Geometry check sheet. Reference: drawing and pictorial views, mm from the part's lowest x, y, z. A direction names the side the tool comes from. Round coordinates to 2 decimals unless told otherwise and drop trailing zeros. Loops run counter-clockwise (first coordinate to the right, second up) from the corner with the lowest first, then second, coordinate; pieces in that order, holes last. Notation, with made-up numbers: (-33.75, 74) -> (-29.75, 74) arc R26 ccw to (-29.75, 103) -> close; hole circle Ø9 at (6.25, 79.5). An arc over 180 degrees is marked (long way). Write item = value, one per line.
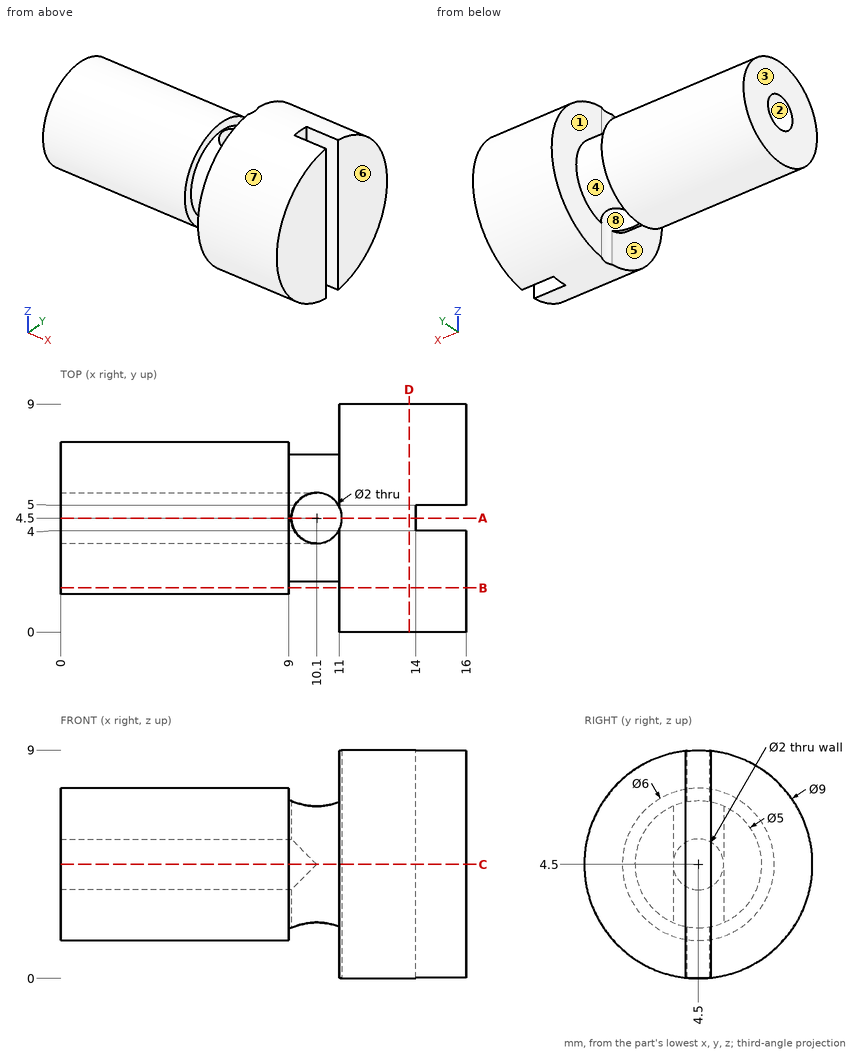
(1) Sectioned sample at B-B, the plane y = 1.75. Record the cut outline in (x, z), and give its area (3 significant figures).
Filled sheet:
outline = (0, 3.3) -> (9, 3.3) -> (9, 5.7) -> (0, 5.7) -> close; (11, 0.94) -> (16, 0.94) -> (16, 8.06) -> (11, 8.06) -> close
area = 57.2 mm2
(2) Draft check along Y on the marked faces 6, 7 and 8. Enter one of: released by +Y, released by -Y, zero draft, split by the parting line, or undercut.
Filled sheet:
face_6 = zero draft
face_7 = split by the parting line
face_8 = undercut
(3) Go/stop test with flat-tipped pins: pin 1 Ø0.5 at (y, z) = (4.5, 4) entering from +X; pin 2 Ø2 at (x, z) = (15, 6.5) entering from -Y; pin 3 Ø1.5 at (x, z) = (2, 5.5) entering from +Y; pin 4 Ø1.8 at (x, y) = (10.1, 4.5) entering from +Z. Record where each tip stops, or that it passes through.
Filled sheet:
pin_1 = 14
pin_2 = 0.11
pin_3 = 7.49
pin_4 = through
(4) Sectioned sample at C-C, the plane z = 4.5. Record the cut outline in (x, y), and give its area (3 significant figures).
Filled sheet:
outline = (0, 1.5) -> (9, 1.5) -> (9, 2) -> (11, 2) -> (11, 0) -> (16, 0) -> (16, 4) -> (14, 4) -> (14, 5) -> (16, 5) -> (16, 9) -> (11, 9) -> (11, 7) -> (9, 7) -> (9, 7.5) -> (0, 7.5) -> (0, 5.5) -> (10.1, 5.5) arc R1 cw to (10.1, 3.5) -> (0, 3.5) -> close
area = 85.2 mm2
(5) Material ranges on probe 1 along Y at (x, z) = (3, 4.5); probe 2 along X at (y, z) = (2, 3.25); probe 3 along X at (y, z) = (2.5, 2), recorded low to high. Write a range as from..to.
Filled sheet:
probe_1 = 1.5..3.5, 5.5..7.5
probe_2 = 0..9, 11..16
probe_3 = 11..16
(6) Sectioned sample at D-D, the plane x = 13.75. Record the cut outline in (y, z), and give its area (3 significant figures).
Filled sheet:
outline = circle Ø9 at (4.5, 4.5)
area = 63.6 mm2
(7) Set-up check for the marked faces 1, 2, 3, 4 and 5: record each of +Z, -Z, +X, -X, +Y, -Y from which the full face is reachable in a straight line by a thin tool's end or side.
Filled sheet:
face_1 = +Y
face_2 = -X
face_3 = +Z, -Z, -X, +Y, -Y
face_4 = none
face_5 = -Y
(8) Sectioned sample at A-A, the plane y = 4.5. Record the cut outline in (x, z), and give its area (3 significant figures).
Filled sheet:
outline = (0, 1.5) -> (9, 1.5) -> (9, 2) -> (9.1, 2) -> (9.1, 3.5) -> (0, 3.5) -> close; (0, 5.5) -> (9.1, 5.5) -> (9.1, 7) -> (9, 7) -> (9, 7.5) -> (0, 7.5) -> close; (11.1, 0) -> (14, 0) -> (14, 9) -> (11.1, 9) -> close
area = 62.4 mm2
